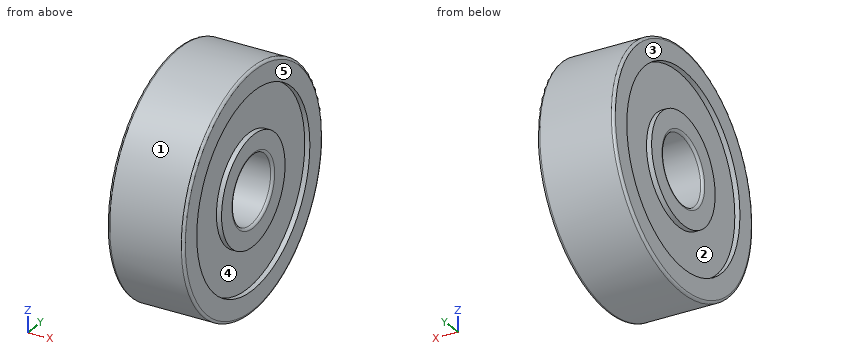
```python
from build123d import *


with BuildPart() as part:
    # Sketch1 → Revolve1 (revolve)
    with BuildSketch(Plane.XY, mode=Mode.PRIVATE) as revolve1_sk:
        with BuildLine():
            Line((0, 11.39), (0.6, 11.39))
            Line((0.6, 11.39), (0.6, 6.4))
            Line((0.6, 6.4), (0, 6.4))
            Line((0, 6.4), (0, 4.3))
            ThreePointArc((0, 4.3), (0.087867966, 4.087867966), (0.3, 4))
            Line((0.3, 4), (8.7, 4))
            ThreePointArc((8.7, 4), (8.912132034, 4.087867966), (9, 4.3))
            Line((9, 4.3), (9, 6.4))
            Line((9, 6.4), (8.4, 6.4))
            Line((8.4, 6.4), (8.4, 11.39))
            Line((8.4, 11.39), (9, 11.39))
            Line((9, 11.39), (9, 13.7))
            ThreePointArc((9, 13.7), (8.912132034, 13.912132034), (8.7, 14))
            Line((8.7, 14), (0.3, 14))
            ThreePointArc((0.3, 14), (0.087867966, 13.912132034), (0, 13.7))
            Line((0, 13.7), (0, 11.39))
        make_face()
    revolve(revolve1_sk.sketch.rotate(Axis((-0.115, 0, 0), (1, 0, 0)), 90), axis=Axis((-0.115, 0, 0), (1, 0, 0)))


solid = part.part
```
The model under review builds one solid part; all positions refer to its coordinate system, in mm. Face numbers are marked on the shaded views. A direction names the side the tool comes from. Give positions to 0.01 mm unless a question says otherwise; leave off trailing zeros. Write each loop counter-clockwise with the first axis right and the second up, starting at its lowest first coordinate (ties: lowest second). Pieces come first, ordered by that corner, then holes. Notation, with made-up numbers: (73.25, 51.25) -> (94.25, 51.25) arc R11 cw to (94.25, 66.25) -> close; hole circle Ø3 at (-21, -26). An arc over 180 degrees is marked (long way). Answer in a Markdown table with one row per item.
1) For L1, parallel to Y at x = 0.35, z = 0; L2, parallel to Y at x = 8.9, z = 0; L3, parallel to Y at x = 5.25, z = 0, list the stretches that pass through material, from the lowest coordinate up. Write a range as [from, to].
Worked answers:
| item | result |
|---|---|
| L1 | [-14, -11.39], [-6.4, -4], [4, 6.4], [11.39, 14] |
| L2 | [-13.92, -11.39], [-6.4, -4.08], [4.08, 6.4], [11.39, 13.92] |
| L3 | [-14, -4], [4, 14] |
2) Mouldability with a two-part tool opening along Y and no side actions: class the marked faces 1, 2 and 3 as +Y half, -Y half, draft (parallel to the pull), parting line (faces both ways), or undercut.
Worked answers:
| item | result |
|---|---|
| face 1 | parting line |
| face 2 | undercut |
| face 3 | draft |
3) Tool access review of the marked faces 4 and 5: name each direction out of +Z, -Z, +X, -X, +Y, -Y from which nothing blocks a thin tool from reaching the whole face with its end or side.
Worked answers:
| item | result |
|---|---|
| face 4 | +X |
| face 5 | +Z, -Z, +X, +Y, -Y |
4) Clearance check with flat-ended pins moving along their axes: P1, Ø2, axis at x = 5, z = -9.5, coming from the -Y side; P2, Ø2, axis at x = 7.5, y = 6, coming from the +Z side; P3, Ø4, axis at x = 8, y = 5.5, coming from the +Z side. State where each tip first meets the part, or that it passes through.
Worked answers:
| item | result |
|---|---|
| P1 | y = -11.12 |
| P2 | z = 13.08 |
| P3 | z = 13.56 |
5) Add section C-C on x = 7.75. State the section outline as (y, z) points, plus the area to 3 significant figures.
Worked answers:
| item | result |
|---|---|
| outline | circle Ø28 at (0, 0); hole circle Ø8 at (0, 0) |
| area | 565 mm² |
